```python
from build123d import *

# Parameters (mm, degrees)
LOWER_ARM_PROFILE_SKETCH_R   = 13.5
LOWER_ARM_PROFILE_SKETCH_R_2 = 7.5
LOWER_CRANK_ARM_DEPTH        = 9
SKETCH1_3_R                  = 7.5
LOWER_ARM_HUB_BOSS_DEPTH     = 6
SHAFT_25_DEPTH               = 75
SHAFT_25_DEPTH_BACK          = 3
SHAFT_25_START               = -9
SHAFT_25_SKETCH_R            = 12.5
SHAFT_25_SKETCH_R_2          = 7.5
SHAFT_COLLAR_SKETCH_R        = 13.5
SHAFT_COLLAR_SKETCH_R_2      = 7.5
SHAFT_COLLAR_DEPTH           = 15
UPPER_START                  = -2
UPPER_ARM_PROFILE_SKETCH_R   = 5
UPPER_CRANK_ARM_DEPTH        = 10


with BuildPart() as part:
    # Lower Arm Profile Sketch → Lower Crank Arm (new, symmetric)
    with BuildSketch(Plane.XY):
        Circle(LOWER_ARM_PROFILE_SKETCH_R)
        Circle(LOWER_ARM_PROFILE_SKETCH_R_2, mode=Mode.SUBTRACT)
    extrude(amount=LOWER_CRANK_ARM_DEPTH, both=True)



with BuildPart() as body_2:
    # Sketch1_3 → Lower Arm Hub Boss (new, symmetric)
    with BuildSketch(Plane.XY):
        with BuildLine():
            ThreePointArc((-45, 13.5), (-58.5, 0), (-45, -13.5))
            Line((-45, -13.5), (0, -13.5))
            ThreePointArc((0, -13.5), (-13.5, 0), (0, 13.5))
            Line((0, 13.5), (-45, 13.5))
        make_face()
        with Locations((-45, 0)):
            Circle(SKETCH1_3_R, mode=Mode.SUBTRACT)
    extrude(amount=LOWER_ARM_HUB_BOSS_DEPTH, both=True)


with BuildPart() as part_1:
    add(part.part)

    add(body_2.part)  # Shaft _25 merges body 2
    # Shaft _25 Sketch → Shaft _25 (add, two sides: drawn at the far end of the back side and taken through both)
    with BuildSketch(Plane.XY.offset(SHAFT_25_START - SHAFT_25_DEPTH_BACK)):
        Circle(SHAFT_25_SKETCH_R)
        Circle(SHAFT_25_SKETCH_R_2, mode=Mode.SUBTRACT)
    extrude(amount=SHAFT_25_DEPTH + SHAFT_25_DEPTH_BACK)

    # Shaft Collar Sketch → Shaft Collar (add)
    with BuildSketch(Plane.XY.offset(66)):
        Circle(SHAFT_COLLAR_SKETCH_R)
        Circle(SHAFT_COLLAR_SKETCH_R_2, mode=Mode.SUBTRACT)
    extrude(amount=-SHAFT_COLLAR_DEPTH)

    # Upper Arm Profile Sketch → Upper Crank Arm (add)
    with BuildSketch(Plane.XY.offset(66).offset(UPPER_START)):
        with BuildLine():
            Line((1.62, 13.402447538), (50.9, 7.445804188))
            ThreePointArc((50.9, 7.445804188), (57.5, 0), (50.9, -7.445804188))
            Line((50.9, -7.445804188), (1.62, -13.402447538))
            ThreePointArc((1.62, -13.402447538), (13.5, 0), (1.62, 13.402447538))
        make_face()
        with Locations((50, 0)):
            Circle(UPPER_ARM_PROFILE_SKETCH_R, mode=Mode.SUBTRACT)
    extrude(amount=-UPPER_CRANK_ARM_DEPTH)


solid = part_1.part
```
The listing builds one solid part. Answer for the finished solid, in the listing's coordinates (mm). A direction names the side the tool comes from. Give positions to 0.01 mm unless a question says otherwise; leave off trailing zeros. Order: outer loops, then holes, each group sorted by start corner. A loop starts at its lowest first (then second) coordinate and runs counter-clockwise, first axis right, second up. Notation, with made-up numbers: (-31.75, 81.25) - (-6.75, 81.25) arc R22 cw to (-6.75, 113.25) - close; hole circle Ø4 at (-26.5, 22.25). An arc over 180 degrees is marked (long way). Use one line per item in the form item = value. Start each with the question number.
(1) Flat-ended cylindrical pins translate along their axes: pin 1 Ø4 at (y, z) = (9.5, 46.5) entering from +X; pin 2 Ø10 at (x, y) = (21, 4) entering from +Z; pin 3 Ø12 at (y, z) = (-5, 17.5) entering from +X; pin 4 Ø13.5 at (x, y) = (-17.5, -2.5) entering from +Z. Find the tip coordinate at first contact, or state that the pin passes through.
(2) A cutting plane is placed at D-D, the plane x = -20.5. Write down the section's boundary in (y, z), then the cut area to 3 significant figures.
(3) Consider line 1 (Y direction, x = 0, z = 33.5); line 2 (Y direction, x = -45, z = 0); line 3 (X direction, y = 5, z = -5). Determine where each line is inside the solid, lowest interval first. Write a range as from..to.
(4) A cutting plane is placed at C-C, the plane z = 45.5. Write down the section's boundary in (x, y).
(5) For faces 4 (the flat face through (6, -6, 66)), 5 (the cylindrical face through (11.923, 3.755, 29.706)), 6 (the flat face through (9, -9, -9)), determine the directions among +Z, -Z, +X, -X, +Y, -Y from which every point of the face is accessible in a straight line to the end or side of a thin tool.
(6) The mould has two halves that part along X. Classify faces 1 (the flat face through (30, 0, 64)), 2 (the cylindrical face through (11.923, 3.755, -10.521)), 3 (the cylindrical face through (-7.493, 0.33, 26.454)): released by +X, released by -X, zero draft, split by the parting line, or undercut.
(7) A cutting plane is placed at A-A, the plane z = -1.5. Write down the section's boundary in (x, y).
(8) A cutting plane is placed at B-B, the plane y = 0. State how many separate pieces and enclosed holes the cut face has, then the cut area to 3 significant figures.
Ans:
q1.pin_1 = 10
q1.pin_2 = 64
q1.pin_3 = 12.5
q1.pin_4 = 66
q2.outline = (-13.5, -6) - (13.5, -6) - (13.5, 6) - (-13.5, 6) - close
q2.area = 324 mm^2
q3.line_1 = -12.5..-7.5, 7.5..12.5
q3.line_2 = -13.5..-7.5, 7.5..13.5
q3.line_3 = -57.54..-50.59, -39.41..-5.59, 5.59..12.54
q4.outline = circle Ø25 at (0, 0); hole circle Ø15 at (0, 0)
q5.face_4 = +Z, +X, -X, +Y, -Y
q5.face_5 = none
q5.face_6 = -Z
q6.face_1 = zero draft
q6.face_2 = split by the parting line
q6.face_3 = undercut
q7.outline = (-45, -13.5) - (0, -13.5) arc R13.5 ccw to (0, 13.5) - (-45, 13.5) arc R13.5 ccw to start; hole circle Ø15 at (-45, 0); hole circle Ø15 at (0, 0)
q8.separate_pieces = 4
q8.enclosed_holes = 0
q8.area = 1,550 mm^2
